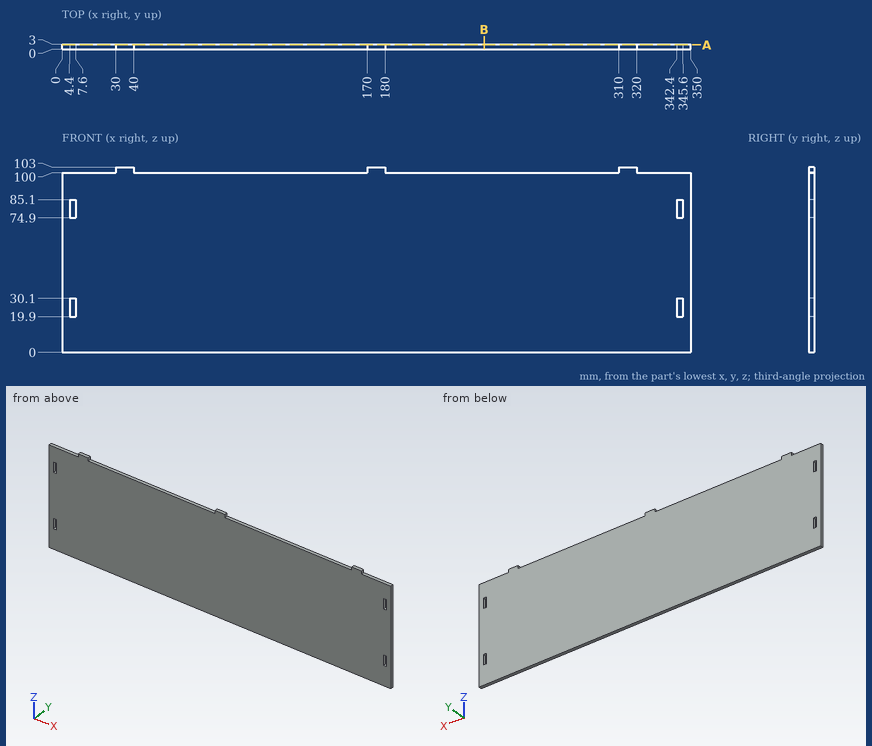
For this review, use the dimensioned drawing (mm, ordinates from the lowest corner) and the shaded views. Coordinates: 2 decimals unless noted, no trailing zeros. Loops run counter-clockwise (first coordinate to the right, second up) from the corner with the lowest first, then second, coordinate; pieces in that order, holes last. Notation, with made-up numbers: (31, 75) - (75, 75) arc R19 cw to (75, 105) - close; hole circle Ø5 at (11.5, 85). An arc over 180 degrees is marked (long way). Use one line per item in the form item = value. Start each with the question number.
1) Take a section at B-B (x = 235). State the section outline as (y, z) points, plus the area to 3 significant figures.
2) For pin 1 (0.9 mm diameter, centred on y = 2, z = 101, fed in from -X); pin 2 (0.9 mm diameter, centred on x = 344.5, y = 1, fed in from -Z); pin 3 (1.5 mm diameter, centred on x = 107.5, y = 0.5, fed in from +Z), all flat-tipped, find the tip position at first contact; note any pin that passes through.
3) Take a section at A-A (y = 2.45). State how many separate pieces and enclosed holes the cut face has, plus the area to 3 significant figures.
4) To check wall thickness, follow probe 1 along X at (y, z) = (2.15, 81); probe 2 along Z at (x, y) = (190, 0.65). State the ranges of each line that lie inside material, in increasing order. Write a range as from..to.
From the geometry:
q1.outline = (0, 0) - (3, 0) - (3, 100) - (0, 100) - close
q1.area = 300 mm2
q2.pin_1 = 30
q2.pin_2 = 0
q2.pin_3 = 100
q3.separate_pieces = 1
q3.enclosed_holes = 4
q3.area = 35,000 mm2
q4.probe_1 = 0..4.4, 7.6..342.4, 345.6..350
q4.probe_2 = 0..100
